Can you work these out from the drawing? Everything is in mm from the part's minimum corner. A direction names the side the tool comes from. Coordinates: 2 decimals unless noted, no trailing zeros. Order: outer loops, then holes, each group sorted by start corner. A loop starts at its lowest first (then second) coordinate and runs counter-clockwise, first axis right, second up. Notation, with made-up numbers: (-28, 60) -> (8, 60) arc R25 ccw to (8, 96) -> close; hole circle Ø5 at (-28.75, 36.5). An arc over 180 degrees is marked (long way). Answer in a Markdown table with one row per item.
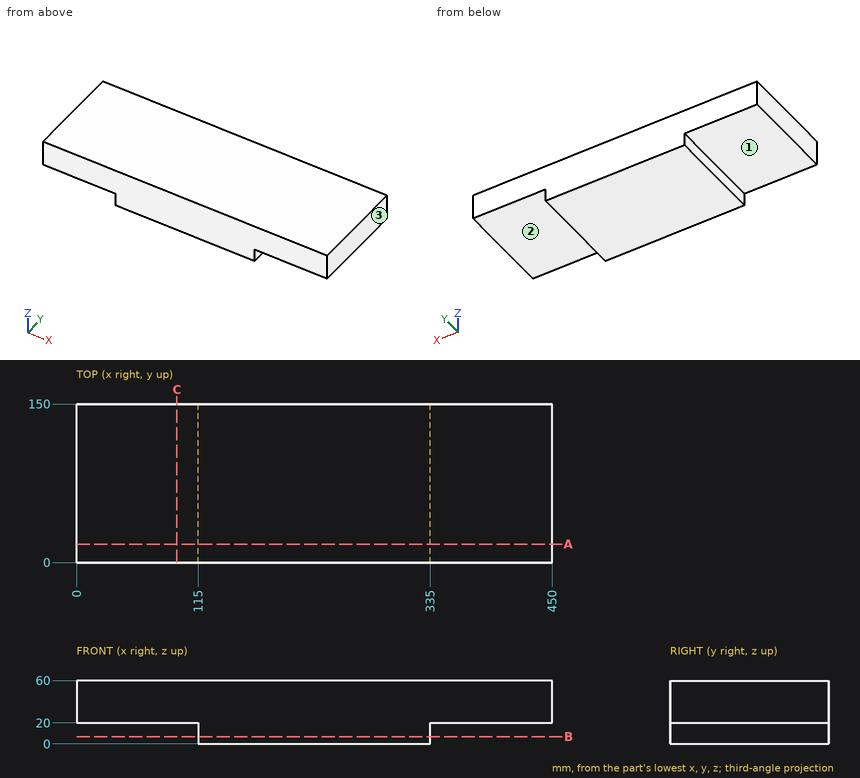
(1) Will these pins go through, and if not, where does the flat tip stop? pin 1 Ø16 at (y, z) = (108.5, 8.5) entering from +X; pin 2 Ø8 at (x, z) = (121.5, 27) entering from -Y; pin 3 Ø5 at (y, z) = (97, 6.5) entering from -X.
Response values:
| item | result |
|---|---|
| pin 1 | x = 335 |
| pin 2 | y = 0 |
| pin 3 | x = 115 |
(2) Suppose I cut it at A-A (y = 17.5). Please give me the cut outline in (x, z).
Response values:
| item | result |
|---|---|
| outline | (0, 20) -> (115, 20) -> (115, 0) -> (335, 0) -> (335, 20) -> (450, 20) -> (450, 60) -> (0, 60) -> close |
(3) On a 3-axis mill with a long thin cutter (end or side, diameter ignored), from which of +Z, -Z, +X, -X, +Y, -Y can I reach the whole of each face in a straight line? I mean the marked faces 1, 2 and 3. Say none if no direction works.
Response values:
| item | result |
|---|---|
| face 1 | -Z, -X, +Y, -Y |
| face 2 | -Z, +X, +Y, -Y |
| face 3 | +Z, -Z, +X, +Y, -Y |
(4) Suppose I cut it at C-C (x = 95). Please give me the cut outline in (y, z), and give its area (3 significant figures).
Response values:
| item | result |
|---|---|
| outline | (0, 20) -> (150, 20) -> (150, 60) -> (0, 60) -> close |
| area | 6,000 mm2 |
(5) Suppose I cut it at B-B (z = 7). Please give me the cut outline in (x, y), and give its area (3 significant figures).
Response values:
| item | result |
|---|---|
| outline | (115, 0) -> (335, 0) -> (335, 150) -> (115, 150) -> close |
| area | 33,000 mm2 |
(6) I need wall thicknesses on line 1 (Z direction, x = 101.5, y = 50); line 2 (X direction, y = 119, z = 6). Which ranges of each line are inside material? Lowest first, please. Write a range as [from, to].
Response values:
| item | result |
|---|---|
| line 1 | [20, 60] |
| line 2 | [115, 335] |
